from build123d import *

# Parameters (mm, degrees)
SKETCH2_R                               = 100
BOSS_EXTRUDE1_DEPTH                     = 12
M10_TAPPED_HOLE1_D                      = 8.5
M10_TAPPED_HOLE1_DEPTH                  = 24.5
M10_TAPPED_HOLE1_TIP                    = 2.553657631
CBORE_FOR_M4_HEX_HEAD_BOLT1_D           = 4.5
CBORE_FOR_M4_HEX_HEAD_BOLT1_DEPTH       = 24.5
CBORE_FOR_M4_HEX_HEAD_BOLT1_CBORE_D     = 8
CBORE_FOR_M4_HEX_HEAD_BOLT1_CBORE_DEPTH = 7
CBORE_FOR_M4_HEX_HEAD_BOLT1_TIP         = 1.351936393
CHAMFER1_SIZE                           = 1


with BuildPart() as part:
    # Sketch2 → Boss-Extrude1 (new body)
    with BuildSketch(Plane(origin=(0, 0, 0), x_dir=(1, 0, 0), z_dir=(0, 1, 0))):
        with Locations(Location((0, 0, 0), (0, 0, 270))):
            Circle(SKETCH2_R)
    extrude(amount=-BOSS_EXTRUDE1_DEPTH)

    # M10 Tapped Hole1
    with Locations(Plane(origin=(-69.282032303, 0, -40), x_dir=(0, 0, 1), z_dir=(0, 1, 0))):
        with Locations((0, 0), (0, 138.564064606), (120, 69.282032303)):
            Hole(M10_TAPPED_HOLE1_D / 2, depth=M10_TAPPED_HOLE1_DEPTH)
            with Locations((0, 0, -(M10_TAPPED_HOLE1_DEPTH + M10_TAPPED_HOLE1_TIP / 2))):  # 118° drill point
                Cone(0, M10_TAPPED_HOLE1_D / 2, M10_TAPPED_HOLE1_TIP, mode=Mode.SUBTRACT)

    # CBORE for M4 Hex Head Bolt1
    with Locations(Plane(origin=(79.64766161, 0, -7.5), x_dir=(0, 0, 1), z_dir=(0, 1, 0))):
        with Locations((0, 0), (15, 0), (15.5, -79.64766161), (-0.5, -79.64766161)):
            CounterBoreHole(CBORE_FOR_M4_HEX_HEAD_BOLT1_D / 2, CBORE_FOR_M4_HEX_HEAD_BOLT1_CBORE_D / 2, CBORE_FOR_M4_HEX_HEAD_BOLT1_CBORE_DEPTH, depth=CBORE_FOR_M4_HEX_HEAD_BOLT1_DEPTH)
            with Locations((0, 0, -(CBORE_FOR_M4_HEX_HEAD_BOLT1_DEPTH + CBORE_FOR_M4_HEX_HEAD_BOLT1_TIP / 2))):  # 118° drill point
                Cone(0, CBORE_FOR_M4_HEX_HEAD_BOLT1_D / 2, CBORE_FOR_M4_HEX_HEAD_BOLT1_TIP, mode=Mode.SUBTRACT)

    # Chamfer1
    chamfer1_edges = [part.edges().sort_by_distance(p)[0] for p in [
        (0, 0, -100),
        (0, -12, -100),
    ]]
    chamfer(chamfer1_edges, length=CHAMFER1_SIZE)


solid = part.part
For this review, take the finished solid that the model builds, in its own axes (mm). A direction names the side the tool comes from. Give positions to 0.01 mm unless a question says otherwise; leave off trailing zeros. Order: outer loops, then holes, each group sorted by start corner. A loop starts at its lowest first (then second) coordinate and runs counter-clockwise, first axis right, second up. Notation, with made-up numbers: (46.25, 20) - (85.25, 20) arc R26 cw to (85.25, 50) - close; hole circle Ø3 at (73, 55). An arc over 180 degrees is marked (long way). Answer as a JSON object with one key per item and string values. Group by question number.
Item 1: Machinability: for faces 1 (the flat face through (-2, -7, -6)), 2 (the cylindrical face through (-71.87, -6.08, -36.63)), which of the approach directions +Z, -Z, +X, -X, +Y, -Y give a long, thin tool a straight path to every point of the face, cutting with its end or side? Answer none if there is none.
Item 2: Take a section at A-A on y = -3.75. Give the boundary of the cut face in (x, z).
Item 3: Clearance check with flat-ended pins moving along their axes: pin 1 Ø1 at (x, y) = (-12.5, -6) entering from +Z; pin 2 Ø2.5 at (x, z) = (79.65, -7.5) entering from +Y; pin 3 Ø7 at (x, z) = (79.65, -7.5) entering from +Y; pin 4 Ø2 at (y, z) = (-7.5, 22) entering from +X. State where each tip first meets the part, or that it passes through.
Item 4: Wall thickness on line 1 along X through (y, z) = (-5.25, 8); line 2 along X through (y, z) = (-7.5, -40); line 3 along X through (y, z) = (-8, 1) (3 decimals): over which ranges is each line inside the solid? List them lowest first.
Item 5: Draft analysis for pull direction X (two halves, no side actions). For faces 3 (the cylindrical face through (77.45, -9.54, -7.01)), 4 (the cylindrical face through (30.04, -5.93, 95.38)), 5 (the flat face through (1, -12, -1)), state which applies: pulls with the +X half, pulls with the -X half, needs draft (parallel to the pull), parting line crosses it, or undercut.
Reported:
{
 "1": {"face 1": "+Y", "face 2": "+Y, -Y"},
 "2": {"outline": "circle Ø200 at (0, 0); hole circle Ø8.5 at (-69.28, -40); hole circle Ø8.5 at (0, 80); hole circle Ø8 at (0, -8); hole circle Ø8 at (0, 8); hole circle Ø8.5 at (69.28, -40); hole circle Ø8 at (79.65, -7.5); hole circle Ø8 at (79.65, 7.5)"},
 "3": {"pin 1": "z = 99.28", "pin 2": "through", "pin 3": "y = -7", "pin 4": "x = 97.77"},
 "4": {"line 1": "-99.68 to -4, 4 to 75.68, 83.62 to 99.68", "line 2": "-91.65 to -73.53, -65.03 to 65.03, 73.53 to 91.65", "line 3": "-99.995 to 99.995"},
 "5": {"face 3": "undercut", "face 4": "parting line crosses it", "face 5": "needs draft"}
}
